```python
from build123d import *

# Parameters (mm, degrees)
SKETCH_1_R                = 60
SKETCH_1_R_2              = 40
EXTRUDE_1_DEPTH           = 15.5
CHAMFER_1_SIZE            = 1
HOLE_WIZARD_1_D           = 6.5
HOLE_WIZARD_1_CBORE_D     = 11
HOLE_WIZARD_1_CBORE_DEPTH = 6.8
SKETCH_7_R                = 42.5
CUT_EXTRUDE_2_DEPTH       = 13
CUT_EXTRUDE_START         = -13
SKETCH_8_R                = 42.5
CUT_EXTRUDE_3_DEPTH       = 13
SKETCH_9_R                = 67.994168063
SKETCH_9_R_2              = 46.5
CUT_EXTRUDE_4_DEPTH       = 10
HOLE_WIZARD_M5_1_D        = 4.2
PATTERN_CIRCULAR_1_COUNT  = 8
SKETCH_10_R               = 6
CUT_EXTRUDE_5_DEPTH       = 10
PATTERN_CIRCULAR_2_COUNT  = 2
PATTERN_CIRCULAR_2_ANGLE  = 45
PATTERN_CIRCULAR_3_COUNT  = 2
PATTERN_CIRCULAR_3_ANGLE  = 45
CHAMFER_2_SIZE            = 1


with BuildPart() as part:
    # 草图1 → 凸台-拉伸1 (new, symmetric)
    with BuildSketch(Plane(origin=(0, 0, 0), x_dir=(1, 0, 0), z_dir=(0, 1, 0))):
        with Locations(Location((0, 0, 0), (0, 0, 270))):
            Circle(SKETCH_1_R)
        with Locations(Location((0, 0, 0), (0, 0, 270))):
            Circle(SKETCH_1_R_2, mode=Mode.SUBTRACT)
    extrude(amount=EXTRUDE_1_DEPTH, both=True)

    # 倒角1
    chamfer_1_edges = [part.edges().sort_by_distance(p)[0] for p in [
        (0, -15.5, -60),
        (0, 15.5, -60),
        (0, -15.5, -40),
        (0, 15.5, -40),
    ]]
    chamfer(chamfer_1_edges, length=CHAMFER_1_SIZE)

    # 打孔尺寸根据内六角圆柱头螺钉的类型1 (through all)
    with Locations(Plane(origin=(-41.126423616, -15.5, 15.006070464), x_dir=(1, 0, 0), z_dir=(0, -1, 0))):
        with Locations((-11.373576384, -15.006070464), (93.626423616, -15.006070464), (41.126423616, -67.506070464), (41.126423616, 37.493929536)):
            hole_wizard_1 = CounterBoreHole(HOLE_WIZARD_1_D / 2, HOLE_WIZARD_1_CBORE_D / 2, HOLE_WIZARD_1_CBORE_DEPTH)

    # 草图7 → 切除-拉伸2 (cut)
    with BuildSketch(Plane(origin=(0, 15.5, 0), x_dir=(1, 0, 0), z_dir=(0, 1, 0))):
        with Locations(Location((0, 0, 0), (0, 0, 270))):
            Circle(SKETCH_7_R)
    extrude(amount=-CUT_EXTRUDE_2_DEPTH, mode=Mode.SUBTRACT)

    # 草图8 → 切除-拉伸3 (cut)
    with BuildSketch(Plane.XZ.offset(15.5).offset(CUT_EXTRUDE_START)):
        with Locations(Location((0, 0, 0), (0, 0, 90))):
            Circle(SKETCH_8_R)
    extrude(amount=CUT_EXTRUDE_3_DEPTH, mode=Mode.SUBTRACT)

    # 草图9 → 切除-拉伸4 (cut)
    with BuildSketch(Plane.XZ.offset(15.5)):
        Circle(SKETCH_9_R)
        with Locations(Location((0, 0, 0), (0, 0, 270))):
            Circle(SKETCH_9_R_2, mode=Mode.SUBTRACT)
    extrude(amount=-CUT_EXTRUDE_4_DEPTH, mode=Mode.SUBTRACT)

    # M5 螺纹孔1 (through all)
    with Locations(Plane(origin=(22.072004657, -5.5, -2.458986171), x_dir=(-1, 0, 0), z_dir=(0, -1, 0))):
        with Locations((-23.594340847, 24.440547066), (-29.239820284, 10.811154044)):
            hole_wizard_m5_1 = Hole(HOLE_WIZARD_M5_1_D / 2)

    # 阵列(圆周)1: M5 螺纹孔1 ×8 about axis
    pattern_circular_1_axis = Axis((0, 0, 0), (0, 1, 0))
    for i in range(1, PATTERN_CIRCULAR_1_COUNT):
        add(hole_wizard_m5_1.rotate(pattern_circular_1_axis, i * 360 / PATTERN_CIRCULAR_1_COUNT), mode=Mode.SUBTRACT)

    # 草图10 → 切除-拉伸5 (cut)
    with BuildSketch(Plane.XZ.offset(5.5)):
        with Locations(Location((0, -52.5, 0), (0, 0, 270))):
            Circle(SKETCH_10_R)
        with Locations(Location((52.5, 0, 0), (0, 0, 270))):
            Circle(SKETCH_10_R)
        with Locations(Location((0, 52.5, 0), (0, 0, 270))):
            Circle(SKETCH_10_R)
        with Locations(Location((-52.5, 0, 0), (0, 0, 270))):
            Circle(SKETCH_10_R)
    cut_extrude_5 = extrude(amount=-CUT_EXTRUDE_5_DEPTH, mode=Mode.SUBTRACT)

    # 阵列(圆周)2: 打孔尺寸根据内六角圆柱头螺钉的类型1 ×2 about axis
    pattern_circular_2_axis = Axis((0, 0, 0), (0, -1, 0))
    for i in range(1, PATTERN_CIRCULAR_2_COUNT):
        add(hole_wizard_1.rotate(pattern_circular_2_axis, i * PATTERN_CIRCULAR_2_ANGLE / (PATTERN_CIRCULAR_2_COUNT - 1)), mode=Mode.SUBTRACT)

    # 阵列(圆周)3: 切除-拉伸5 ×2 about axis
    pattern_circular_3_axis = Axis((0, 0, 0), (0, -1, 0))
    for i in range(1, PATTERN_CIRCULAR_3_COUNT):
        add(cut_extrude_5.rotate(pattern_circular_3_axis, i * PATTERN_CIRCULAR_3_ANGLE / (PATTERN_CIRCULAR_3_COUNT - 1)), mode=Mode.SUBTRACT)

    # 倒角2
    chamfer_2_edges = [part.edges().sort_by_distance(p)[0] for p in [
        (0, 15.5, -42.5),
        (0, -15.5, -42.5),
    ]]
    chamfer(chamfer_2_edges, length=CHAMFER_2_SIZE)


solid = part.part
```
Input: part model. Units: mm. Frame: model coordinates. A direction names the side the tool comes from. Coordinates: 2 decimals unless noted, no trailing zeros. Write each loop counter-clockwise with the first axis right and the second up, starting at its lowest first coordinate (ties: lowest second). Pieces come first, ordered by that corner, then holes. Notation, with made-up numbers: (88, 45) -> (103, 45) arc R18 ccw to (103, 62) -> close; hole circle Ø11 at (85, 68.25). An arc over 180 degrees is marked (long way). Write each question's results on one line, items separated by ' | '.
Item 1: Material intervals for probe 1 along X at (y, z) = (7, -38); probe 2 along Z at (x, y) = (-36, 6); probe 3 along X at (y, z) = (-3, 45), sorted ascending.
Conclusion:
probe 1: x = -46.43 to -40.25, -33.99 to -19.03, 19.03 to 33.99, 40.25 to 46.43 | probe 2: z = -48 to -40.17, -34.07 to -22.59, 22.59 to 34.07, 40.17 to 48 | probe 3: x = -39.69 to -28.89, -24.91 to 24.91, 28.89 to 39.69
Item 2: Section query A-A on y = -1. Count the separate pieces of the cut face and the enclosed holes in it, plus the area to 3 significant figures.
Conclusion:
separate pieces: 1 | enclosed holes: 25 | area: 5,160 mm^2
Item 3: Set-up query: faces 1 (the cylindrical face through (-25.861, 8.584, -33.727)), 2 (the flat face through (-37, 4.5, 33)), 3 (the cylindrical face through (45.21, 5.15, -24.85)). Return all of +Z, -Z, +X, -X, +Y, -Y with unobstructed straight access to the full face (end or side cutting, diameter ignored); none if empty.
Conclusion:
face 1: +Y | face 2: -Y | face 3: +Y, -Y
Item 4: Pin query (flat end, axial travel): pin 1 Ø3.5 at (x, z) = (-53, 2) entering from -Y; pin 2 Ø8 at (x, y) = (19, -10) entering from +Z; pin 3 Ø5 at (x, z) = (42.5, 39.5) entering from -Y. Return the tip coordinate at first contact, or that it passes through.
Conclusion:
pin 1: stops at y = 4.5 | pin 2: stops at z = 44.01 | pin 3: stops at y = -5.5
Item 5: Section query B-B on y = -8.5. Return loops of the section in (x, z).
Conclusion:
outline: circle Ø93 at (0, 0); hole circle Ø85 at (0, 0)
